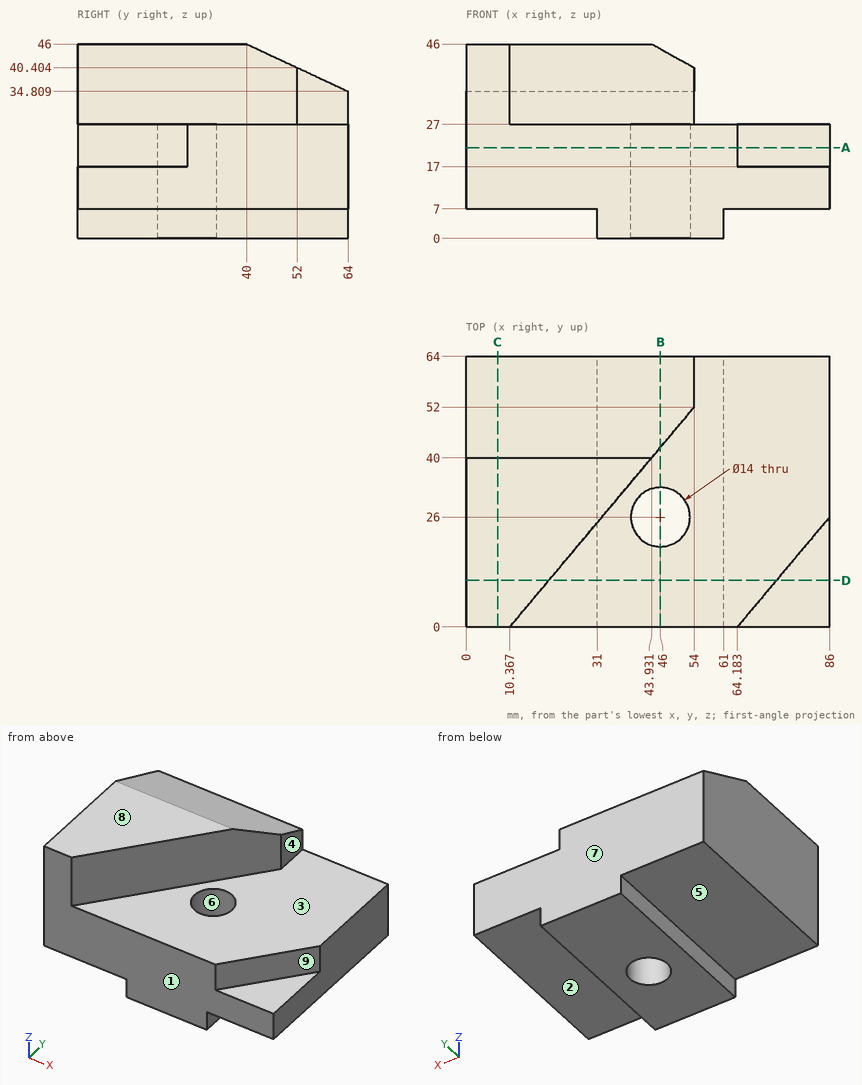
The figure shows three views and two pictorial views of one solid part (mm, origin at its lowest corner). Answer the questions. A direction names the side the tool comes from. Coordinates: 2 decimals unless noted, no trailing zeros. Order: outer loops, then holes, each group sorted by start corner. A loop starts at its lowest first (then second) coordinate and runs counter-clockwise, first axis right, second up.
Q1. A cutting plane is placed at C-C, the plane x = 7.5. Write down the section's boundary in (y, z), and give its area (3 significant figures).
Q2. Consider line 1 (Y direction, x = 46, z = 17); line 2 (Z direction, x = 21.5, y = 25.5); line 3 (X direction, y = 10, z = 5). Determine where each line is inside the solid, lowest interval first.
Q3. A cutting plane is placed at D-D, the plane y = 11. Write down the section's boundary in (x, z).
Q4. For a pull along Y with two mould halves and no side action, classify the marked faces 6, 7, 8 and 9 as pulls with the +Y half, pulls with the -Y half, needs draft (parallel to the pull), parting line crosses it, or undercut.
Q5. A cutting plane is placed at B-B, the plane x = 46. Write down the section's boundary in (y, z), and give its area (3 significant figures).
Q6. Which of the six approach directions +Z, -Z, +X, -X, +Y, -Y give full straight-line access (tool end or side, diameter ignored) to the marked faces 1, 2, 3, 4 and 5?
Q7. A cutting plane is placed at A-A, the plane z = 21.5. Write down the section's boundary in (x, y), and give its area (3 significant figures).
Q8. Given P1, Ø8, axis at y = 23, z = 21, coming from the -X side; P2, Ø2, axis at y = 27.5, z = 3, coming from the -X side; P3, Ø3, axis at x = 66.5, y = 33.5, coming from the +Z side; P4, Ø13, axis at y = 60, z = 35, coming from the +X side, each flat-ended and moving along its own axis, determine where each tip first touches the part or whether it passes through.
Answers follow:
1. outline: (0, 7) - (64, 7) - (64, 34.81) - (40, 46) - (0, 46) - close
1. area: 2,360 mm2
2. line 1: y = 0 to 19, 33 to 64
2. line 2: z = 7 to 46
2. line 3: x = 31 to 61
3. outline: (0, 7) - (31, 7) - (31, 0) - (61, 0) - (61, 7) - (86, 7) - (86, 17) - (73.41, 17) - (73.41, 27) - (19.6, 27) - (19.6, 46) - (0, 46) - close
4. face 6: undercut
4. face 7: pulls with the +Y half
4. face 8: needs draft
4. face 9: pulls with the -Y half
5. outline: (0, 0) - (19, 0) - (19, 27) - (0, 27) - close; (33, 0) - (64, 0) - (64, 34.81) - (42.47, 44.85) - (42.47, 27) - (33, 27) - close
5. area: 1,630 mm2
6. face 1: +Z, -Z, +X, -X, -Y
6. face 2: -Z, +X, +Y, -Y
6. face 3: +Z, +X, -Y
6. face 4: +Z, +X, +Y, -Y
6. face 5: -Z, -X, +Y, -Y
7. outline: (0, 0) - (64.18, 0) - (86, 26) - (86, 64) - (0, 64) - close; hole circle Ø14 at (46, 26)
7. area: 5,070 mm2
8. P1: stops at x = 0
8. P2: stops at x = 31
8. P3: stops at z = 27
8. P4: stops at x = 54
